For this review, take the finished solid that the model builds, in its own axes (mm). Face numbers are marked on the shaded views. A direction names the side the tool comes from. Coordinates: 2 decimals unless noted, no trailing zeros. Order: outer loops, then holes, each group sorted by start corner. A loop starts at its lowest first (then second) coordinate and runs counter-clockwise, first axis right, second up. Notation, with made-up numbers: M 67.25,44 L 96.25,44 A34 ccw 96.25,77 Z; hole C -14,-23 d8. An arc over 180 degrees is marked long. Use CSV: the item, a comma, the result in double quotes.
```python
from build123d import *

# Parameters (mm, degrees)
EXTRUDE_387_DEPTH = 10
FILLET_1280_R     = 0.6


with BuildPart() as part:
    # 草图1 → Extrude 387 (new body)
    with BuildSketch(Plane(origin=(0, 0, 0), x_dir=(0, 0, -1), z_dir=(1, 0, 0))):
        Polygon((12, 6.92820323), (12, -6.92820323), (0, -13.856406461), (-12, -6.92820323), (-12, 6.92820323), (0, 13.856406461), align=None)
    extrude(amount=EXTRUDE_387_DEPTH)

    # 草图2 → 凸台-旋转1 (revolve)
    with BuildSketch(Plane.XY, mode=Mode.PRIVATE) as revolve_1_sk:
        Polygon((0, 0), (50, 0), (50, 6.268), (50, 8), (12, 8), (0, 8), align=None)
    revolve(revolve_1_sk.sketch.rotate(Axis((0, 0, 0), (1, 0, 0)), 90), axis=Axis((0, 0, 0), (1, 0, 0)))

    # 草图3 → 切除-旋转1 (revolve, cut)
    with BuildSketch(Plane.XY):
        Polygon((0, 12), (3.958548116, 18.856406461), (3.958548116, 23.856406461), (-10, 23.856406461), (-10, 12), align=None)
    revolve(axis=Axis((0, 0, 0), (1, 0, 0)), mode=Mode.SUBTRACT)

    # 草图4 → 切除-旋转3 (revolve, cut)
    with BuildSketch(Plane.XY, mode=Mode.PRIVATE) as cut_revolve_3_sk:
        Polygon((10, 11.245), (9.2, 11.706880215), (9.2, 13.856406461), (10, 13.856406461), align=None)
    revolve(cut_revolve_3_sk.sketch.rotate(Axis((0, 0, 0), (1, 0, 0)), 90), axis=Axis((0, 0, 0), (1, 0, 0)), mode=Mode.SUBTRACT)

    # Fillet 1280
    fillet_1280_edges = [part.edges().sort_by_distance(p)[0] for p in [
        (10, 0, -8),
    ]]
    fillet(fillet_1280_edges, radius=FILLET_1280_R)


solid = part.part
```
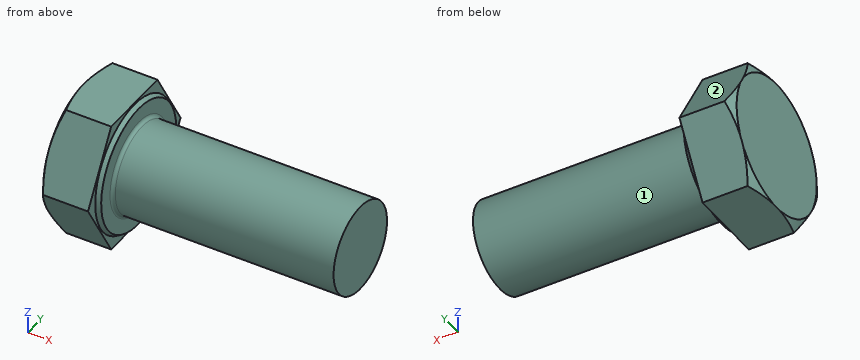
Item 1: Add section A-A on x = 27.5. State the section outline as (y, z) points, and give its area (3 significant figures).
Solutions:
outline,"C 0,0 d16"
area,"201 mm^2"
Item 2: Clearance check with flat-ended pins moving along their axes: pin 1 Ø6 at (x, z) = (45, 9.5) entering from +Y; pin 2 Ø1 at (x, z) = (11.5, -2.5) entering from +Y; pin 3 Ø10 at (x, z) = (38, 2.5) entering from -Y. State where each tip first meets the part, or that it passes through.
Solutions:
pin 1,"y = 4.66"
pin 2,"y = 7.75"
pin 3,"y = -8"
Item 3: For the marked faces 1 and 2, list the 3-axis set-ups (+Z, -Z, +X, -X, +Y, -Y) from which the entire face can be reached by the end or side of a thin tool; tool diameter is ignored.
Solutions:
face 1,"+X"
face 2,"+Z, +X, -X, +Y"
Item 4: To check wall thickness, follow line 1 along X through (y, z) = (-8.25, -5.75); line 2 along Y through (x, z) = (13, -4); line 3 along Y through (x, z) = (4, -6). State the ranges of each line that lie inside material, in increasing order. Write a range as [from, to].
Solutions:
line 1,"[0, 10]"
line 2,"[-6.93, 6.93]"
line 3,"[-10.39, 10.39]"
